Check sheet for the modelled part. Datum: model origin and axes. Units: mm. Round coordinates to 2 decimals unless told otherwise and drop trailing zeros. Order: outer loops, then holes, each group sorted by start corner. A loop starts at its lowest first (then second) coordinate and runs counter-clockwise, first axis right, second up.
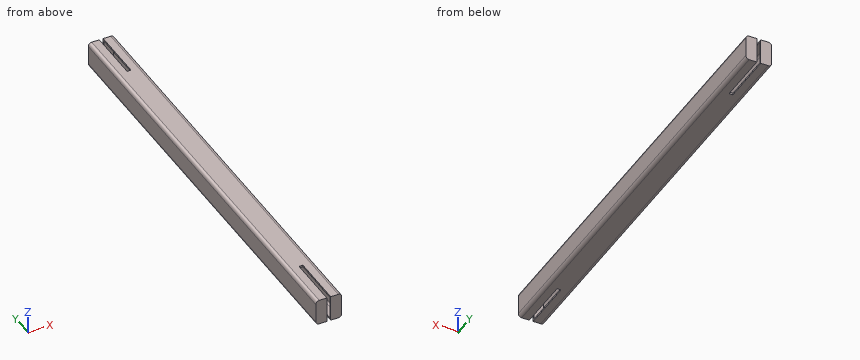
```python
from build123d import *

# Parameters (mm, degrees)
BOSS_EXTRUDE1_DEPTH     = 998
CUT_EXTRUDE1_DEPTH      = 1001.251968256
CUT_EXTRUDE1_DEPTH_BACK = 1001.251968256
SKETCH2_W               = 9
SKETCH2_H               = 244
SKETCH3_W               = 21.5
SKETCH3_H               = 52
BOSS_EXTRUDE2_DEPTH     = 4
SKETCH4_W               = 21.5
SKETCH4_H               = 52
BOSS_EXTRUDE3_DEPTH     = 4


with BuildPart() as part:
    # Sketch1 → Boss-Extrude1 (new body)
    with BuildSketch(Plane(origin=(0, 0, 0), x_dir=(1, 0, 0), z_dir=(0, 1, 0))):
        with BuildLine():
            Line((-22, -30), (22, -30))
            ThreePointArc((22, -30), (27.656854249, -27.656854249), (30, -22))
            Line((30, -22), (30, 22))
            ThreePointArc((30, 22), (27.656854249, 27.656854249), (22, 30))
            Line((22, 30), (-22, 30))
            ThreePointArc((-22, 30), (-27.656854249, 27.656854249), (-30, 22))
            Line((-30, 22), (-30, -22))
            ThreePointArc((-30, -22), (-27.656854249, -27.656854249), (-22, -30))
        make_face()
        with BuildLine():
            Line((-22, 26), (22, 26))
            ThreePointArc((22, 26), (24.828427125, 24.828427125), (26, 22))
            Line((26, 22), (26, -22))
            ThreePointArc((26, -22), (24.828427125, -24.828427125), (22, -26))
            Line((22, -26), (-22, -26))
            ThreePointArc((-22, -26), (-24.828427125, -24.828427125), (-26, -22))
            Line((-26, -22), (-26, 22))
            ThreePointArc((-26, 22), (-24.828427125, 24.828427125), (-22, 26))
        make_face(mode=Mode.SUBTRACT)
    extrude(amount=BOSS_EXTRUDE1_DEPTH)

    # Sketch2 → Cut-Extrude1 (cut, two sides: drawn at the far end of the back side and taken through both)
    with BuildSketch(Plane.XY.offset(30).offset(-CUT_EXTRUDE1_DEPTH_BACK)):
        with Locations((0, 998)):
            Rectangle(SKETCH2_W, SKETCH2_H)
        Rectangle(SKETCH2_W, SKETCH2_H)
    extrude(amount=CUT_EXTRUDE1_DEPTH + CUT_EXTRUDE1_DEPTH_BACK, mode=Mode.SUBTRACT)

    # Sketch3 → Boss-Extrude2 (add)
    with BuildSketch(Plane(origin=(0, 998, 0), x_dir=(1, 0, 0), z_dir=(0, 1, 0))):
        with Locations((-15.25, 0)):
            Rectangle(SKETCH3_W, SKETCH3_H)
        with Locations((15.25, 0)):
            Rectangle(SKETCH3_W, SKETCH3_H)
    extrude(amount=-BOSS_EXTRUDE2_DEPTH)

    # Sketch4 → Boss-Extrude3 (add)
    with BuildSketch(Plane.XZ):
        with Locations((-15.25, 0)):
            Rectangle(SKETCH4_W, SKETCH4_H)
        with Locations((15.25, 0)):
            Rectangle(SKETCH4_W, SKETCH4_H)
    extrude(amount=-BOSS_EXTRUDE3_DEPTH)


solid = part.part
```
Item 1: Sectioned sample at A-A (z = -1). Record the cut outline in (x, y).
Answer:
outline: (-30, 0) - (-4.5, 0) - (-4.5, 4) - (-26, 4) - (-26, 994) - (-4.5, 994) - (-4.5, 998) - (-30, 998) - close; (4.5, 0) - (30, 0) - (30, 998) - (4.5, 998) - (4.5, 994) - (26, 994) - (26, 4) - (4.5, 4) - close
Item 2: Sectioned sample at C-C (y = 918). Record the cut outline in (x, z), and give its area (3 significant figures).
Answer:
outline: (-30, -22) arc R8 ccw to (-22, -30) - (-4.5, -30) - (-4.5, -26) - (-22, -26) arc R4 cw to (-26, -22) - (-26, 22) arc R4 cw to (-22, 26) - (-4.5, 26) - (-4.5, 30) - (-22, 30) arc R8 ccw to (-30, 22) - close; (4.5, -30) - (22, -30) arc R8 ccw to (30, -22) - (30, 22) arc R8 ccw to (22, 30) - (4.5, 30) - (4.5, 26) - (22, 26) arc R4 cw to (26, 22) - (26, -22) arc R4 cw to (22, -26) - (4.5, -26) - close
area: 783 mm2
Item 3: Go/stop test with flat-tipped pins: P1, Ø4.5, axis at x = 2, z = 28.5, coming from the -Y side; P2, Ø3, axis at x = 1.5, z = -28.5, coming from the +Y side. Record where each tip stops, or that it passes through.
Answer:
P1: stops at y = 122
P2: stops at y = 876
Item 4: Scan lines: line 1 along Y through (x, z) = (8, 19.5); line 2 along X through (y, z) = (681, -7). Record each from-to range of solid material in increasing order.
Answer:
line 1: y = 0 to 4, 994 to 998
line 2: x = -30 to -26, 26 to 30
Item 5: Sectioned sample at B-B (y = 355). Record the cut outline in (x, z), and give its area (3 significant figures).
Answer:
outline: (-30, -22) arc R8 ccw to (-22, -30) - (22, -30) arc R8 ccw to (30, -22) - (30, 22) arc R8 ccw to (22, 30) - (-22, 30) arc R8 ccw to (-30, 22) - close; hole (-26, -22) arc R4 ccw to (-22, -26) - (22, -26) arc R4 ccw to (26, -22) - (26, 22) arc R4 ccw to (22, 26) - (-22, 26) arc R4 ccw to (-26, 22) - close
area: 855 mm2
